```python
from build123d import *

# Parameters (mm, degrees)
BOSS_EXTRUDE1_DEPTH = 6
CHAMFER1_SIZE       = 15


with BuildPart() as part:
    # Sketch1 → Boss-Extrude1 (new body)
    with BuildSketch(Plane.XY):
        Polygon((0, 60), (0, 0), (60, 0), (60, 10), (10, 60), align=None)
    extrude(amount=BOSS_EXTRUDE1_DEPTH)

    # Chamfer1
    chamfer1_edges = [part.edges().sort_by_distance(p)[0] for p in [
        (0, 0, 3),
    ]]
    chamfer(chamfer1_edges, length=CHAMFER1_SIZE)


solid = part.part
```
Design review of the part built by this model. Coordinates are the model's own, in mm. Give positions to 0.01 mm unless a question says otherwise; leave off trailing zeros. Loops run counter-clockwise (first coordinate to the right, second up) from the corner with the lowest first, then second, coordinate; pieces in that order, holes last. Notation, with made-up numbers: (82.25, -8.5) -> (123.25, -8.5) arc R19 cw to (123.25, 15.5) -> close; hole circle Ø7 at (-12, 47.25). An arc over 180 degrees is marked (long way). One line per item, written item: value.
Q1. We need section C-C on y = 23.5. Give the boundary of the cut face in (x, z).
Numbers:
outline: (0, 0) -> (46.5, 0) -> (46.5, 6) -> (0, 6) -> close
Q2. For pin 1 Ø2 at (x, z) = (23, 1.5) entering from +Y, flat-tipped, find the tip position at first contact; note if it passes through.
Numbers:
pin 1: stops at y = 48
Q3. We need section A-A on x = 45.5. Give the boundary of the cut face in (y, z).
Numbers:
outline: (0, 0) -> (24.5, 0) -> (24.5, 6) -> (0, 6) -> close
Q4. For L1, parallel to Y at x = 33, z = 2.5; L2, parallel to X at y = 26, z = 4.9; L3, parallel to Y at x = 37, z = 3.25, list the stretches that pass through material, from the lowest coordinate up.
Numbers:
L1: y = 0 to 37
L2: x = 0 to 44
L3: y = 0 to 33
Q5. We need section B-B on z = 3.4. Give the boundary of the cut face in (x, y), and give its area (3 significant figures).
Numbers:
outline: (0, 15) -> (15, 0) -> (60, 0) -> (60, 10) -> (10, 60) -> (0, 60) -> close
area: 2,240 mm^2
